Work out the finished part from the listing and answer in its coordinate system (mm). Round coordinates to 2 decimals unless told otherwise and drop trailing zeros. Order: outer loops, then holes, each group sorted by start corner. A loop starts at its lowest first (then second) coordinate and runs counter-clockwise, first axis right, second up. Notation, with made-up numbers: (18, 74) -> (67, 74) arc R31 cw to (67, 113) -> close; hole circle Ø1 at (36.5, 16.5). An arc over 180 degrees is marked (long way). Use a Markdown table: item, result. Add a question column.
Item 1: Find the intervals of material crossed by L1, parallel to Y at x = 0, z = 3.65; L2, parallel to Y at x = 0, z = 9.5; L3, parallel to X at y = -254, z = 8, in increasing order. Write a range as [from, to].
Item 2: Flat-ended cylindrical pins translate along their axes: P1, Ø5, axis at x = -9.5, z = 7, coming from the +Y side; P2, Ø1, axis at x = -11, z = 11.5, coming from the -Y side; P3, Ø14.5, axis at x = 0, y = 130, coming from the +Z side. Find the tip coordinate at first contact, or state that the pin passes through.
Item 3: A cutting plane is placed at A-A, the plane z = 12.5. Determine the outline of the cut face in (x, y), plus the area to 3 significant figures.
Item 4: A cutting plane is placed at B-B, the plane x = -15. Determine the outline of the cut face in (y, z).
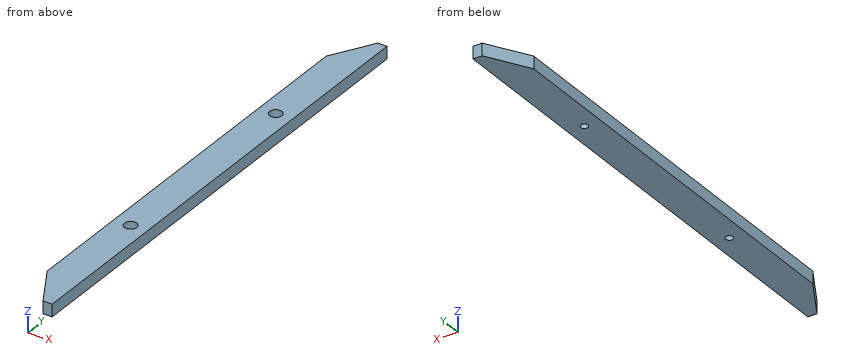
from build123d import *

# Parameters (mm, degrees)
SKETCH_1_W                = 40
SKETCH_1_H                = 600
EXTRUDE_1_DEPTH           = 15
HOLE_WIZARD_1_D           = 9
HOLE_WIZARD_1_CBORE_D     = 15
HOLE_WIZARD_1_CBORE_DEPTH = 9
CHAMFER_1_SIZE            = 50
CHAMFER_1_SIZE2           = 28.867513459


with BuildPart() as part:
    # 草图1 → 凸台-拉伸1 (new body)
    with BuildSketch(Plane.XY):
        Rectangle(SKETCH_1_W, SKETCH_1_H)
    extrude(amount=EXTRUDE_1_DEPTH)

    # 打孔尺寸(%根据)内六角圆柱头螺钉的类型1 (through all)
    with Locations(Plane.XY.offset(15)):
        with Locations((0, -130), (0, 130)):
            CounterBoreHole(HOLE_WIZARD_1_D / 2, HOLE_WIZARD_1_CBORE_D / 2, HOLE_WIZARD_1_CBORE_DEPTH)

    # 倒角1
    chamfer_1_edges = [part.edges().sort_by_distance(p)[0] for p in [
        (-20, 300, 7.5),
        (-20, -300, 7.5),
    ]]
    chamfer_1_side = [part.faces().sort_by_distance(p)[0] for p in [
        (-20, 0, 7.5),
    ]]
    chamfer(chamfer_1_edges, length=CHAMFER_1_SIZE, length2=CHAMFER_1_SIZE2, reference=chamfer_1_side[0])


solid = part.part
Reported:
| question | item | result |
|---|---|---|
| 1 | L1 | [-284.64, -134.5], [-125.5, 125.5], [134.5, 284.64] |
| 1 | L2 | [-284.64, -137.5], [-122.5, 122.5], [137.5, 284.64] |
| 1 | L3 | [-17.69, 20] |
| 2 | P1 | y = 272.52 |
| 2 | P2 | y = -266.45 |
| 2 | P3 | z = 6 |
| 3 | outline | (-20, -250) -> (8.87, -300) -> (20, -300) -> (20, 300) -> (8.87, 300) -> (-20, 250) -> close; hole circle Ø15 at (0, -130); hole circle Ø15 at (0, 130) |
| 3 | area | 22,200 mm² |
| 4 | outline | (-258.66, 0) -> (258.66, 0) -> (258.66, 15) -> (-258.66, 15) -> close |
